Part model, mm, in its own coordinate system. Give positions to 0.01 mm unless a question says otherwise; leave off trailing zeros. Order: outer loops, then holes, each group sorted by start corner. A loop starts at its lowest first (then second) coordinate and runs counter-clockwise, first axis right, second up. Notation, with made-up numbers: (60, 24) - (86, 24) arc R6 cw to (86, 30) - close; hole circle Ø10 at (-18, 55). An arc over 180 degrees is marked (long way). One line per item, written item: value.
```python
from build123d import *

# Parameters (mm, degrees)
SKETCH1_R           = 5
BOSS_EXTRUDE1_DEPTH = 4


with BuildPart() as part:
    # Sketch1 → Boss-Extrude1 (new body)
    with BuildSketch(Plane.XY):
        with BuildLine():
            Line((0, 0), (50, 0))
            Line((50, 0), (42.27924078, 23.16227766))
            ThreePointArc((42.27924078, 23.16227766), (38.639510646, 28.112421852), (32.792407799, 30))
            Line((32.792407799, 30), (17.207592201, 30))
            ThreePointArc((17.207592201, 30), (11.360489354, 28.112421852), (7.72075922, 23.16227766))
            Line((7.72075922, 23.16227766), (0, 0))
        make_face()
        with Locations((25, 20)):
            Circle(SKETCH1_R, mode=Mode.SUBTRACT)
    extrude(amount=BOSS_EXTRUDE1_DEPTH)


solid = part.part
```
1) Cut at B-B, the plane z = 1.2. Give the cut face in (x, y), then the cut area to 3 significant figures.
Outcome:
outline: (0, 0) - (50, 0) - (42.28, 23.16) arc R10 ccw to (32.79, 30) - (17.21, 30) arc R10 ccw to (7.72, 23.16) - close; hole circle Ø10 at (25, 20)
area: 1,100 mm^2
2) Cut at A-A, the plane x = 25. Give the cut face in (y, z).
Outcome:
outline: (0, 0) - (15, 0) - (15, 4) - (0, 4) - close; (25, 0) - (30, 0) - (30, 4) - (25, 4) - close
3) Pin check, flat tips, straight feed: pin 1 (4 mm diameter, centred on x = 44.5, y = 23, fed in from +Z); pin 2 (2 mm diameter, centred on y = 11.5, z = 3, fed in from -X); pin 3 (2 mm diameter, centred on y = 23.5, z = 0.5, fed in from +X). Stop position of each tip, or through.
Outcome:
pin 1: passes through
pin 2: stops at x = 3.5
pin 3: stops at x = 42.5
4) Drill centre lines: line 1 along Y through (x, z) = (25, 2.3); line 2 along Y through (x, z) = (23, 3.85); line 3 along X through (y, z) = (18, 0.6). Where is each one in solid material? Low to high. Write a range as from..to.
Outcome:
line 1: y = 0..15, 25..30
line 2: y = 0..15.42, 24.58..30
line 3: x = 6..20.42, 29.58..44
5) Mould opens along X. For faces 1 (the cylindrical face through (21, 17, 2)), 2 (the flat face through (25, 0, 2)), 3 (the flat face through (4, 12, 2)) say: released by +X, released by -X, zero draft, split by the parting line, or undercut.
Outcome:
face 1: undercut
face 2: zero draft
face 3: released by -X
6) Cut at D-D, the plane y = 9. Give the cut face in (x, z), then the cut area to 3 significant figures.
Outcome:
outline: (3, 0) - (47, 0) - (47, 4) - (3, 4) - close
area: 176 mm^2
7) Cut at C-C, the plane y = 19.5. Give the cut face in (x, z).
Outcome:
outline: (6.5, 0) - (20.03, 0) - (20.03, 4) - (6.5, 4) - close; (29.97, 0) - (43.5, 0) - (43.5, 4) - (29.97, 4) - close
